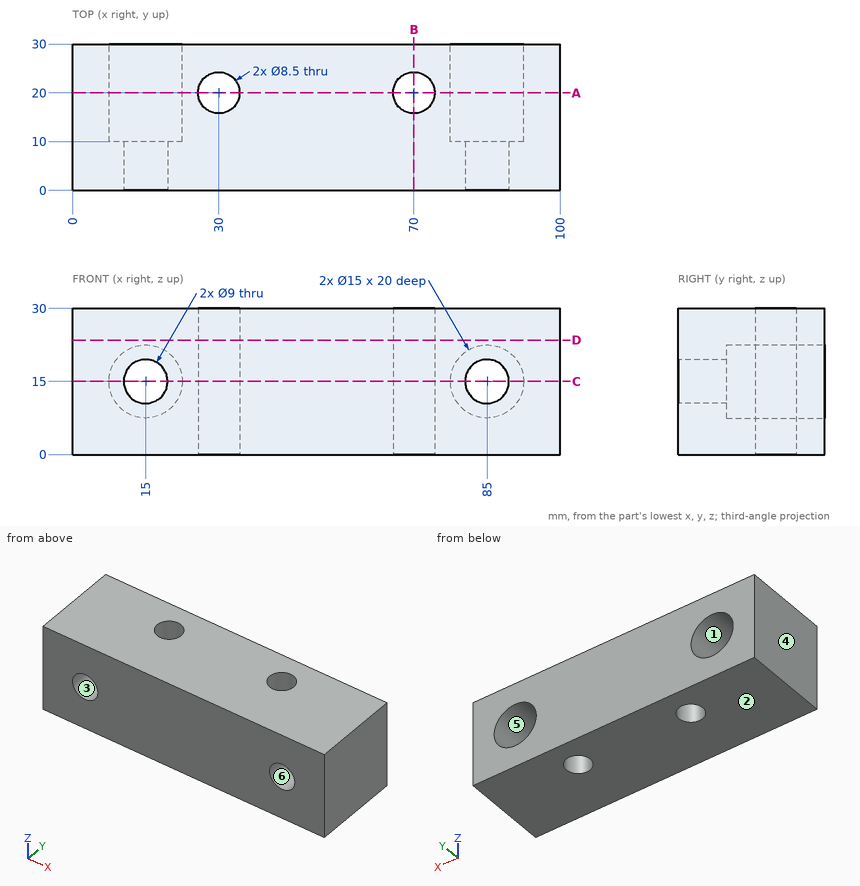
Study the drawing (mm; zero at the part's minimum x, y, z) and answer. A direction names the side the tool comes from. Give positions to 0.01 mm unless a question says otherwise; leave off trailing zeros. Loops run counter-clockwise (first coordinate to the right, second up) from the corner with the lowest first, then second, coordinate; pieces in that order, holes last. Notation, with made-up numbers: M 53,6.5 L 98,6.5 A31 cw 98,42.5 Z; hole C 27.5,56 d6. An arc over 180 degrees is marked long. One line per item, written item: value.
1. Section C-C on z = 15 is taken. Determine the outline of the cut face in (x, y).
Found:
outline: M 0,0 L 10.5,0 L 10.5,10 L 7.5,10 L 7.5,30 L 0,30 Z; M 19.5,0 L 80.5,0 L 80.5,10 L 77.5,10 L 77.5,30 L 22.5,30 L 22.5,10 L 19.5,10 Z; M 89.5,0 L 100,0 L 100,30 L 92.5,30 L 92.5,10 L 89.5,10 Z; hole C 30,20 d8.5; hole C 70,20 d8.5
2. For the marked faces 5 and 6, determine the directions among +Z, -Z, +X, -X, +Y, -Y from which every point of the face is accessible in a straight line to the end or side of a thin tool.
Found:
face 5: +Y
face 6: +Y, -Y
3. Each of these flat-tipped pins is pushed along its axis until it touches: P1, Ø8, axis at x = 85, z = 15, coming from the -Y side; P2, Ø7.5, axis at x = 85.5, z = 18.5, coming from the +Y side. Where does it stop, or does it pass through?
Found:
P1: through
P2: y = 10
4. For a pull along Z with two mould halves and no side action, classify the marked faces 1, 2, 3 and 4 as pulls with the +Z half, pulls with the -Z half, needs draft (parallel to the pull), parting line crosses it, or undercut.
Found:
face 1: undercut
face 2: pulls with the -Z half
face 3: undercut
face 4: needs draft
5. Find the intervals of material crossed by probe 1 along X at (y, z) = (3.25, 16); probe 2 along X at (y, z) = (19, 2.25); probe 3 along Y at (x, z) = (85, 20), in increasing order.
Found:
probe 1: 0 to 10.61, 19.39 to 80.61, 89.39 to 100
probe 2: 0 to 25.87, 34.13 to 65.87, 74.13 to 100
probe 3: 0 to 10
6. Section B-B on x = 70 is taken. Determine the outline of the cut face in (y, z), plus the area to 3 significant figures.
Found:
outline: M 0,0 L 15.75,0 L 15.75,30 L 0,30 Z; M 24.25,0 L 30,0 L 30,30 L 24.25,30 Z
area: 645 mm^2
7. Section A-A on y = 20 is taken. Determine the outline of the cut face in (x, z).
Found:
outline: M 0,0 L 25.75,0 L 25.75,30 L 0,30 Z; M 34.25,0 L 65.75,0 L 65.75,30 L 34.25,30 Z; M 74.25,0 L 100,0 L 100,30 L 74.25,30 Z; hole C 15,15 d15; hole C 85,15 d15
8. Section D-D on z = 23.5 is taken. Determine the outline of the cut face in (x, y), plus the area to 3 significant figures.
Found:
outline: M 0,0 L 100,0 L 100,30 L 0,30 Z; hole C 30,20 d8.5; hole C 70,20 d8.5
area: 2,890 mm^2
